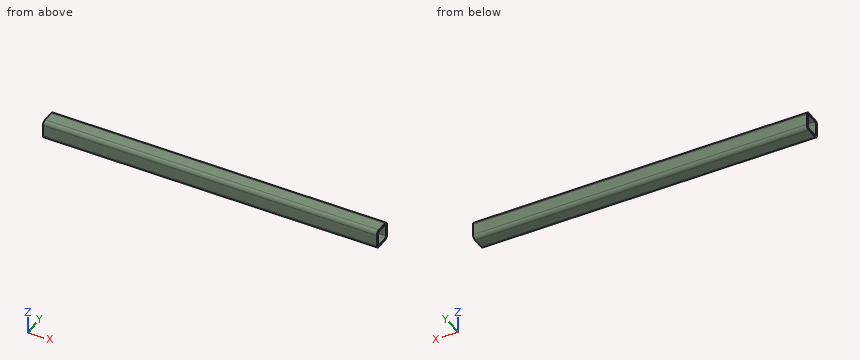
from build123d import *

# Parameters (mm, degrees)
SQUARE_TUBE_40_X_40_X_4_1_DEPTH = 720


with BuildPart() as part:
    # Sketch1 → Square Tube 40 X 40 X 4(1) (new body)
    with BuildSketch(Plane.YZ.offset(-1000)):
        with BuildLine():
            Line((-12, -20), (12, -20))
            ThreePointArc((12, -20), (17.656854249, -17.656854249), (20, -12))
            Line((20, -12), (20, 12))
            ThreePointArc((20, 12), (17.656854249, 17.656854249), (12, 20))
            Line((12, 20), (-12, 20))
            ThreePointArc((-12, 20), (-17.656854249, 17.656854249), (-20, 12))
            Line((-20, 12), (-20, -12))
            ThreePointArc((-20, -12), (-17.656854249, -17.656854249), (-12, -20))
        make_face()
        with BuildLine():
            Line((-12, -16), (12, -16))
            ThreePointArc((12, -16), (14.828427125, -14.828427125), (16, -12))
            Line((16, -12), (16, 12))
            ThreePointArc((16, 12), (14.828427125, 14.828427125), (12, 16))
            Line((12, 16), (-12, 16))
            ThreePointArc((-12, 16), (-14.828427125, 14.828427125), (-16, 12))
            Line((-16, 12), (-16, -12))
            ThreePointArc((-16, -12), (-14.828427125, -14.828427125), (-12, -16))
        make_face(mode=Mode.SUBTRACT)
    extrude(amount=SQUARE_TUBE_40_X_40_X_4_1_DEPTH)


solid = part.part
Geometry check sheet. Reference: the model listing, model coordinates, mm. Coordinates: 2 decimals unless noted, no trailing zeros. Order: outer loops, then holes, each group sorted by start corner. A loop starts at its lowest first (then second) coordinate and runs counter-clockwise, first axis right, second up. Notation, with made-up numbers: (41, 26) - (50, 26) arc R22 ccw to (50, 58) - close; hole circle Ø10 at (66, 36). An arc over 180 degrees is marked (long way). Answer in a Markdown table with one row per item. Add a question column.
1) Material ranges on line 1 along Z through (x, y) = (-414, -2.5); line 2 along Y through (x, z) = (-737.5, 14), recorded low to high. Write a range as [from, to].
2) Cross-section at A-A, the plane x = -675. Record the cut outline in (y, z), then the cut area to 3 significant figures.
3) Cross-section at B-B, the plane y = 2. Record the cut outline in (x, z).
Check result:
| question | item | result |
|---|---|---|
| 1 | line 1 | z = [-20, -16], [16, 20] |
| 1 | line 2 | y = [-19.75, -15.46], [15.46, 19.75] |
| 2 | outline | (-20, -12) arc R8 ccw to (-12, -20) - (12, -20) arc R8 ccw to (20, -12) - (20, 12) arc R8 ccw to (12, 20) - (-12, 20) arc R8 ccw to (-20, 12) - close; hole (-16, -12) arc R4 ccw to (-12, -16) - (12, -16) arc R4 ccw to (16, -12) - (16, 12) arc R4 ccw to (12, 16) - (-12, 16) arc R4 ccw to (-16, 12) - close |
| 2 | area | 535 mm² |
| 3 | outline | (-1000, -20) - (-280, -20) - (-280, -16) - (-1000, -16) - close; (-1000, 16) - (-280, 16) - (-280, 20) - (-1000, 20) - close |
